Verification items for the finished model (mm, model axes). A direction names the side the tool comes from. Round coordinates to 2 decimals unless told otherwise and drop trailing zeros. Write each loop counter-clockwise with the first axis right and the second up, starting at its lowest first coordinate (ties: lowest second). Pieces come first, ordered by that corner, then holes.
from build123d import *

# Parameters (mm, degrees)
V_BLOCK_PROFILE_SKETCH_R = 22.5
V_BLOCK_BODY_DEPTH       = 25
CROSS_HOLE_SKETCH_R      = 6.164856296
CROSS_HOLE_DEPTH         = 60


with BuildPart() as part:
    # V-Block Profile Sketch → V-Block Body (new, symmetric)
    with BuildSketch(Plane.XY):
        with BuildLine():
            Line((-40.000071852, 52.924513188), (-40.000071852, 92.924513188))
            Line((-40.000071852, 92.924513188), (-30.000071852, 92.924513188))
            Line((-30.000071852, 92.924513188), (-6.165, 72.924513188))
            Line((-6.165, 72.924513188), (6.164856296, 72.924513188))
            Line((6.164856296, 72.924513188), (29.999928148, 92.924513188))
            Line((29.999928148, 92.924513188), (39.999928148, 92.924513188))
            Line((39.999928148, 92.924513188), (39.999928148, 52.924513188))
            ThreePointArc((39.999928148, 52.924513188), (27.538857009, 41.183981608), (28.726666617, 24.104535363))
            ThreePointArc((28.726666617, 24.104535363), (0, -37.5), (-28.726666617, 24.104535363))
            ThreePointArc((-28.726666617, 24.104535363), (-27.538910641, 41.184022764), (-40.000071852, 52.924513188))
        make_face()
        Circle(V_BLOCK_PROFILE_SKETCH_R, mode=Mode.SUBTRACT)
    extrude(amount=V_BLOCK_BODY_DEPTH, both=True)

    # Cross Hole Sketch → Cross Hole (cut)
    with BuildSketch(Plane(origin=(0, 72.924513188, 0), x_dir=(1, 0, 0), z_dir=(0, 1, 0))):
        with Locations(Location((0, 0, 0), (0, 0, 270))):
            Circle(CROSS_HOLE_SKETCH_R)
    extrude(amount=-CROSS_HOLE_DEPTH, mode=Mode.SUBTRACT)


solid = part.part
Q1. Sectioned sample at B-B (y = 0). Enter the section's corners in (x, z).
Recorded:
outline: (-37.5, -25) - (-22.5, -25) - (-22.5, 25) - (-37.5, 25) - close; (22.5, -25) - (37.5, -25) - (37.5, 25) - (22.5, 25) - close
Q2. Sectioned sample at C-C (x = -33.5). Enter the section's corners in (y, z).
Recorded:
outline: (-16.85, -25) - (16.85, -25) - (16.85, 25) - (-16.85, 25) - close; (49.38, -25) - (92.92, -25) - (92.92, 25) - (49.38, 25) - close
Q3. Sectioned sample at A-A (x = 0). Enter the section's corners in (y, z), plus the area to 3 significant figures.
Recorded:
outline: (-37.5, -25) - (-22.5, -25) - (-22.5, 25) - (-37.5, 25) - close; (22.5, -25) - (72.92, -25) - (72.92, -6.16) - (22.5, -6.16) - close; (22.5, 6.16) - (72.92, 6.16) - (72.92, 25) - (22.5, 25) - close
area: 2,650 mm2
Q4. Depth check by flat-ended pin: P1, Ø6, axis at x = -2, z = -4.5, coming from the +Y side; P2, Ø1, axis at x = 32, z = -11.5, coming from the -Y side; P3, Ø3, axis at y = 49.5, z = -13, coming from the +X side. Enter the tip coordinate at first touch or a pass-through.
Recorded:
P1: stops at y = 72.92
P2: stops at y = -20.35
P3: stops at x = 35.79
Q5. Release check for a two-part mould opening along Y. For faces 4 (the flat face through (40, 73, 0)), 5 (the cylindrical face through (-27.45, 40.95, 0.35)), 6 (the flat face through (-18.249, 83.065, 0.35)) record: released by +Y, released by -Y, zero draft, split by the parting line, or undercut.
Recorded:
face 4: zero draft
face 5: undercut
face 6: released by +Y
Q6. Material ranges on line 1 along Z through (x, y) = (0, 58); line 2 along Y through (x, z) = (28, -15); line 3 along X through (y, z) = (36.5, 0), recorded low to high.
Recorded:
line 1: z = -25 to -6.16, 6.16 to 25
line 2: y = -24.94 to 25.53, 42.27 to 91.25
line 3: x = -26.33 to -6.16, 6.16 to 26.33
Q7. Sectioned sample at D-D (z = -18). Enter the section's corners in (x, y) (3 decimals), plus the area to 3 significant figures.
Recorded:
outline: (-40, 52.925) arc R20 cw to (-28.727, 24.105) arc R37.5 ccw (long way) to (28.727, 24.105) arc R20 cw to (40, 52.925) - (40, 92.925) - (30, 92.925) - (6.165, 72.925) - (-6.165, 72.925) - (-30, 92.925) - (-40, 92.925) - close; hole circle Ø45 at (0, 0)
area: 6,430 mm2
Q8. Tool access check on faces 1 (the flat face through (17.916, 82.785, 0.35)), 2 (the flat face through (1, 29, 25)), 3 (the cylindrical face through (-6.018, 47.64, -1.336)). Record the directions out of +Z, -Z, +X, -X, +Y, -Y that give a thin tool (end or side, any length) a straight path to the whole face; none if there is none.
Recorded:
face 1: +Z, -Z, +Y
face 2: +Z, +X, -X, +Y, -Y
face 3: +Y
